from build123d import *

# Parameters (mm, degrees)
SKETCH1_R                = 15
BOSS_EXTRUDE1_DEPTH      = 8.5
CUT_EXTRUDE1_DEPTH       = 23.852789764
CUT_EXTRUDE1_DEPTH_BACK  = 23.852789764
SKETCH2_R                = 3
BOSS_EXTRUDE2_REACH      = 41.016
BOSS_EXTRUDE2_END_RADIUS = 15
SKETCH3_R                = 5
SKETCH3_R_2              = 3
BOSS_EXTRUDE3_START      = 3
SKETCH4_R                = 8.5
SKETCH4_R_2              = 3
BOSS_EXTRUDE3_DEPTH      = 3
FILLET1_R                = 0.5


with BuildPart() as part:
    # Sketch1 → Boss-Extrude1 (new, symmetric)
    with BuildSketch(Plane.XY):
        Circle(SKETCH1_R)
    extrude(amount=BOSS_EXTRUDE1_DEPTH, both=True)

    # Sketch2 → Cut-Extrude1 (cut, two sides: drawn at the far end of the back side and taken through both)
    with BuildSketch(Plane(origin=(0, 0, 0), x_dir=(1, 0, 0), z_dir=(0, 1, 0)).offset(-CUT_EXTRUDE1_DEPTH_BACK)):
        with Locations(Location((0, 0, 0), (0, 0, 270))):
            Circle(SKETCH2_R)
    extrude(amount=CUT_EXTRUDE1_DEPTH + CUT_EXTRUDE1_DEPTH_BACK, mode=Mode.SUBTRACT)

    # Boss-Extrude2: up to this cylinder (the profile starts outside it)
    boss_extrude2_end = Plane(origin=(0, 0, -4.858579), z_dir=(0, 0, -1)) * Cylinder(BOSS_EXTRUDE2_END_RADIUS, 113.032, mode=Mode.PRIVATE)
    # Sketch3 → Boss-Extrude2 (add, up to the surface)
    with BuildSketch(Plane(origin=(0, 20, 0), x_dir=(1, 0, 0), z_dir=(0, 1, 0)), mode=Mode.PRIVATE) as boss_extrude2_sk1:
        with Locations(Location((0, 0, 0), (0, 0, 270))):
            Circle(SKETCH3_R)
        with Locations(Location((0, 0, 0), (0, 0, 270))):
            Circle(SKETCH3_R_2, mode=Mode.SUBTRACT)
    boss_extrude2_tool1 = extrude(boss_extrude2_sk1.sketch, amount=-BOSS_EXTRUDE2_REACH, mode=Mode.PRIVATE) - boss_extrude2_end
    add(boss_extrude2_tool1.solids().sort_by_distance((0, 20, -4.858579))[0])

    # Sketch4 → Boss-Extrude3 (add)
    with BuildSketch(Plane(origin=(0, 20, 0), x_dir=(1, 0, 0), z_dir=(0, 1, 0)).offset(BOSS_EXTRUDE3_START)):
        with Locations(Location((0, 0, 0), (0, 0, 270))):
            Circle(SKETCH4_R)
        with Locations(Location((0, 0, 0), (0, 0, 270))):
            Circle(SKETCH4_R_2, mode=Mode.SUBTRACT)
    extrude(amount=-BOSS_EXTRUDE3_DEPTH)

    # Fillet1
    fillet1_edges = [part.edges().sort_by_distance(p)[0] for p in [
        (0, 23, -8.5),
    ]]
    fillet(fillet1_edges, radius=FILLET1_R)


solid = part.part
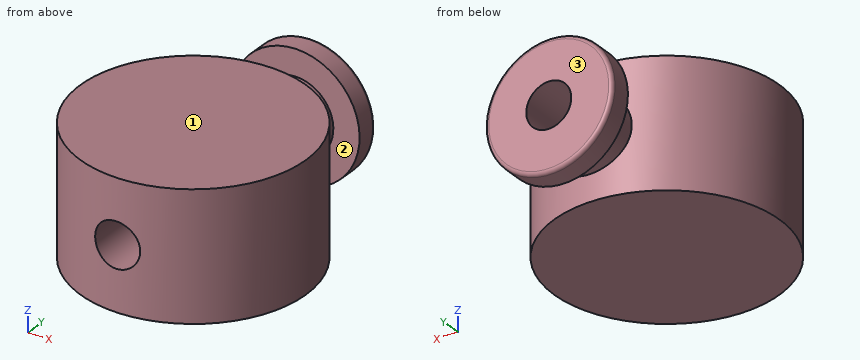
Read the model definition and answer for the solid it produces. Units are mm, in the model's axes. Face numbers are marked on the shaded views. Give positions to 0.01 mm unless a question says otherwise; leave off trailing zeros. Write each loop counter-clockwise with the first axis right and the second up, starting at its lowest first coordinate (ties: lowest second). Pieces come first, ordered by that corner, then holes. Notation, with made-up numbers: (-7, 51) - (35, 51) arc R16 ccw to (35, 82) - close; hole circle Ø9 at (84, -8.75). An arc over 180 degrees is marked (long way). Use CSV: the item, a comma, the result in double quotes. Start each with the question number.
Item 1: Consider line 1 (Z direction, x = 0, y = 4); line 2 (Z direction, x = 0, y = 17). Determine where each line is inside the solid, lowest interval first.
Item 2: Flat-ended cylindrical pins translate along their axes: P1, Ø3, axis at y = 16, z = 0, coming from the -X side; P2, Ø5.5, axis at x = 0, z = 0, coming from the +Y side; P3, Ø5, axis at y = 8.5, z = -0.5, coming from the +X side; P4, Ø3, axis at y = 14, z = -5, coming from the -X side. Find the tip coordinate at first contact, or state that the pin passes through.
Item 3: The part is cut by section D-D, the plane x = 12. Give the vertices of the cut face in (y, z), and give its area (3 significant figures).
Item 4: The part is cut by section C-C, the plane z = 0. Give the vertices of the cut face in (x, y).
Item 5: The mould has two halves that part along Y. Classify the marked faces 1, 2 and 3: pulls with the +Y half, pulls with the -Y half, needs draft (parallel to the pull), parting line crosses it, or undercut.
Item 6: The part is cut by section A-A, the plane x = 0. Give the vertices of the cut face in (y, z).
Item 7: The part is cut by section B-B, the plane y = 0. Give the vertices of the cut face in (x, z).
Taken from the geometry:
1,line 1,"-8.5 to -3, 3 to 8.5"
1,line 2,"-5 to -3, 3 to 5"
2,P1,"x = -5"
2,P2,"through"
2,P3,"x = 13.75"
2,P4,"x = -8.29"
3,outline,"(-9, -8.5) - (9, -8.5) - (9, 8.5) - (-9, 8.5) - close"
3,area,"306 mm2"
4,outline,"(-8.5, 20) - (-5, 20) - (-5, 14.14) arc R15 ccw to (-3, -14.7) - (-3, 23) - (-8, 23) arc R0.5 ccw to (-8.5, 22.5) - close; (3, -14.7) arc R15 ccw to (5, 14.14) - (5, 20) - (8.5, 20) - (8.5, 22.5) arc R0.5 ccw to (8, 23) - (3, 23) - close"
5,face 1,"needs draft"
5,face 2,"undercut"
5,face 3,"pulls with the +Y half"
6,outline,"(-15, -8.5) - (15, -8.5) - (15, -5) - (20, -5) - (20, -8.5) - (22.5, -8.5) arc R0.5 ccw to (23, -8) - (23, -3) - (-15, -3) - close; (-15, 3) - (23, 3) - (23, 8) arc R0.5 ccw to (22.5, 8.5) - (20, 8.5) - (20, 5) - (15, 5) - (15, 8.5) - (-15, 8.5) - close"
7,outline,"(-15, -8.5) - (15, -8.5) - (15, 8.5) - (-15, 8.5) - close; hole circle Ø6 at (0, 0)"
